from build123d import *

# Parameters (mm, degrees)
M4_TAPPED_HOLE1_D     = 3.3
M4_TAPPED_HOLE1_DEPTH = 10.1
M4_TAPPED_HOLE1_TIP   = 0.991420021


with BuildPart() as part:
    # Sketch1 → Revolve1 (revolve)
    with BuildSketch(Plane(origin=(0, 0, 0), x_dir=(0, 0, -1), z_dir=(1, 0, 0))):
        with BuildLine():
            Line((0, 0), (10.725, 0))
            Line((10.725, 0), (10.725, 2.45))
            ThreePointArc((10.725, 2.45), (7.382093902, 3.853488302), (6, 7.205296327))
            Line((6, 7.205296327), (6, 13))
            Line((6, 13), (13.200228011, 21))
            Line((13.200228011, 21), (13.200228011, 21.5))
            ThreePointArc((13.200228011, 21.5), (12.098891552, 23.906448602), (10.25, 25.8))
            Line((10.25, 25.8), (0, 25.8))
            Line((0, 25.8), (0, 0))
        make_face()
    revolve(axis=Axis((0, 0, 0), (0, 1, 0)))

    # M4 Tapped Hole1
    with Locations(Plane(origin=(0, 0, 0), x_dir=(-1, 0, 0), z_dir=(0, -1, 0))):
        with Locations((0, 0)):
            Hole(M4_TAPPED_HOLE1_D / 2, depth=M4_TAPPED_HOLE1_DEPTH)
            with Locations((0, 0, -(M4_TAPPED_HOLE1_DEPTH + M4_TAPPED_HOLE1_TIP / 2))):  # 118° drill point
                Cone(0, M4_TAPPED_HOLE1_D / 2, M4_TAPPED_HOLE1_TIP, mode=Mode.SUBTRACT)


solid = part.part
Model file for the job. Use its own axes, mm. A direction names the side the tool comes from. Coordinates: 2 decimals unless noted, no trailing zeros. Order: outer loops, then holes, each group sorted by start corner. A loop starts at its lowest first (then second) coordinate and runs counter-clockwise, first axis right, second up. Notation, with made-up numbers: (56.5, 86) -> (114.5, 86) arc R24 cw to (114.5, 115) -> close; hole circle Ø10 at (-17.75, -38). An arc over 180 degrees is marked (long way). Return JSON: item names as keys, results as strings. Group by question number.
Item 1: Flat gauge pins, fed straight in: P1, Ø1.5, axis at x = 0.5, y = 4, coming from the +Z side; P2, Ø1.5, axis at x = -2.5, y = 22.5, coming from the +Z side; P3, Ø1.5, axis at x = 2, z = -2, coming from the -Y side; P4, Ø12, axis at y = 6, z = -8.5, coming from the +X side. Where does each tip first touch, or does it go through?
Item 2: Saw through at B-B on y = 18.75. Write the cut outline in (x, z), then the cut area to 3 significant figures.
Item 3: Wall check: line 1 along Z through (x, y) = (0, 7.5); line 2 along Y through (x, z) = (0.25, 6.75); line 3 along Y through (x, z) = (-8.75, -3). Give the ranges that are in metal, low to high. Write a range as [from, to].
Item 4: Saw through at A-A on y = 4. Write the cut outline in (x, z), then the cut area to 3 significant figures.
Item 5: Pull direction X, two halves, no side cores. Call faces 1 (the conical face through (0.1, 10.9, 0.3)), 2 (the conical face through (5.72, 13.5, -2.98)), 3 (the flat face through (0, 0, 2)): pulls with the +X half, pulls with the -X half, needs draft (parallel to the pull), parting line crosses it, or undercut.
Item 6: Tool access for faces 4 (the cylindrical face through (0, 10, 6)), 5 (the cylindrical face through (-7.248, 1.242, 7.905)), 6 (the cylindrical face through (-3.965, 21.254, -12.591)): list every direction of +Z, -Z, +X, -X, +Y, -Y with a clear straight run to the whole face (end or side of a thin tool).
Values found:
{
 "1": {"P1": "stops at z = 8.1", "P2": "stops at z = 12.93", "P3": "stops at y = 0", "P4": "stops at x = 10.08"},
 "2": {"outline": "circle Ø22.35 at (0, 0)", "area": "392 mm2"},
 "3": {"line 1": "z = [-6, -1.65], [1.65, 6]", "line 2": "y = [0, 4.63], [13.84, 25.8]", "line 3": "y = [0, 2.69], [16.61, 25.8]"},
 "4": {"outline": "circle Ø14.49 at (0, 0); hole circle Ø3.3 at (0, 0)", "area": "156 mm2"},
 "5": {"face 1": "undercut", "face 2": "parting line crosses it", "face 3": "needs draft"},
 "6": {"face 4": "none", "face 5": "-Y", "face 6": "+Y, -Y"}
}
